Check sheet for the modelled part. Datum: model origin and axes. Units: mm. Coordinates: 2 decimals unless noted, no trailing zeros. Loops run counter-clockwise (first coordinate to the right, second up) from the corner with the lowest first, then second, coordinate; pieces in that order, holes last. Notation, with made-up numbers: M -4,73.25 L 38,73.25 A35 ccw 38,112.25 Z; hole C 51,78 d6. An arc over 180 degrees is marked long. Use CSV: the item, a comma, the result in double quotes. Start each with the question number.
(1) Section check C-C on x = 83.5. Record the cut outline in (y, z).
(2) Section check B-B on y = 2.25. Record the cut outline in (x, z).
(3) Section check A-A on x = 0. Record the cut outline in (y, z), and give its area (3 significant figures).
(4) Scan lines: line 1 (X direction, y = -1.5, z = 90); line 2 (Z direction, x = 81, y = 3.5). Record each from-to range of solid material in increasing order.
(5) Go/stop test with a flat-tipped pin: pin 1 Ø12 at (x, z) = (-80, -90) entering from +Y. Record where the tip stops, or that it passes through.
(6) Draft check along Z on faces 1 (the cylindrical face through (-86.654, 0.07, -86.539)), 2 (the cylindrical face through (-94.297, 0.07, 103.986)), 3 (the flat face through (-1, 5, -2)). Enter one of: pulls with the +Z half, pulls with the -Z half, needs draft (parallel to the pull), parting line crosses it, or undercut.
from build123d import *

# Parameters (mm, degrees)
SKETCH1_W            = 200
SKETCH1_H            = 220
BOSS_EXTRUDE1_DEPTH  = 5
SKETCH2_R            = 7.5
CUT_EXTRUDE1_DEPTH   = 10
LPATTERN1_COUNT      = 2
LPATTERN1_PITCH      = 180
LPATTERN1_COUNT_DIR2 = 3
LPATTERN1_PITCH_DIR2 = 80
FILLET1_R            = 20


with BuildPart() as part:
    # Sketch1 → Boss-Extrude1 (new, symmetric)
    with BuildSketch(Plane(origin=(0, 0, 0), x_dir=(1, 0, 0), z_dir=(0, 1, 0))):
        Rectangle(SKETCH1_W, SKETCH1_H)
    extrude(amount=BOSS_EXTRUDE1_DEPTH, both=True)

    # Sketch2 → Cut-Extrude1 (cut)
    with BuildSketch(Plane(origin=(0, 5, 0), x_dir=(1, 0, 0), z_dir=(0, 1, 0))):
        with Locations(Location((80, 90, 0), (0, 0, 270))):
            Circle(SKETCH2_R)
    cut_extrude1 = extrude(amount=-CUT_EXTRUDE1_DEPTH, mode=Mode.SUBTRACT)

    # LPattern1: Cut-Extrude1 2 × 3
    with Locations(*[(-j * LPATTERN1_PITCH_DIR2, 0, i * LPATTERN1_PITCH) for i in range(LPATTERN1_COUNT) for j in range(LPATTERN1_COUNT_DIR2) if (i, j) != (0, 0)]):
        add(cut_extrude1, mode=Mode.SUBTRACT)

    # Fillet1
    fillet1_edges = [part.edges().sort_by_distance(p)[0] for p in [
        (100, 0, 110),
        (-100, 0, 110),
        (-100, 0, -110),
        (100, 0, -110),
    ]]
    fillet(fillet1_edges, radius=FILLET1_R)


solid = part.part
Outcome:
1,outline,"M -5,-109.69 L 5,-109.69 L 5,-96.63 L -5,-96.63 Z; M -5,-83.37 L 5,-83.37 L 5,83.37 L -5,83.37 Z; M -5,96.63 L 5,96.63 L 5,109.69 L -5,109.69 Z"
2,outline,"M -100,-90 A20 ccw -80,-110 L 80,-110 A20 ccw 100,-90 L 100,90 A20 ccw 80,110 L -80,110 A20 ccw -100,90 Z; hole C -80,-90 d15; hole C -80,90 d15; hole C 0,-90 d15; hole C 0,90 d15; hole C 80,-90 d15; hole C 80,90 d15"
3,outline,"M -5,-110 L 5,-110 L 5,-97.5 L -5,-97.5 Z; M -5,-82.5 L 5,-82.5 L 5,82.5 L -5,82.5 Z; M -5,97.5 L 5,97.5 L 5,110 L -5,110 Z"
3,area,"1,900 mm²"
4,line 1,"x = -100 to -87.5, -72.5 to -7.5, 7.5 to 72.5, 87.5 to 100"
4,line 2,"z = -109.97 to -97.43, -82.57 to 82.57, 97.43 to 109.97"
5,pin 1,"passes through"
6,face 1,"undercut"
6,face 2,"pulls with the +Z half"
6,face 3,"needs draft"
